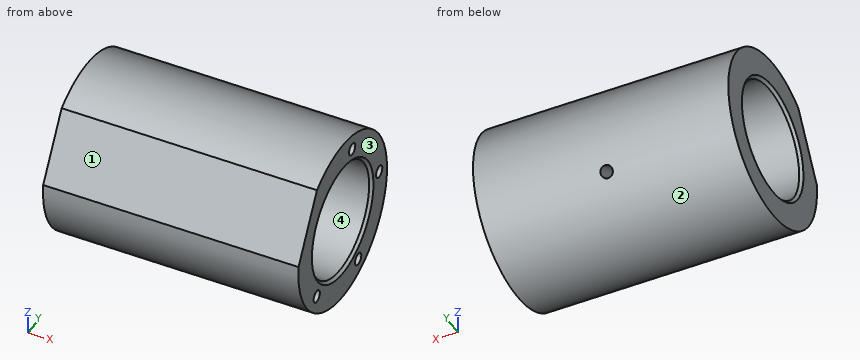
from build123d import *

# Parameters (mm, degrees)
SKETCH1_R               = 60.5
SKETCH1_R_2             = 40
BOSS_EXTRUDE1_DEPTH     = 90
CUT_EXTRUDE1_DEPTH      = 125.179305844
CUT_EXTRUDE1_DEPTH_BACK = 125.179305844
SKETCH6_W               = 4.25
SKETCH6_H               = 82.644536929
M10_TAPPED_HOLE2_D      = 8.5
M10_TAPPED_HOLE2_DEPTH  = 32
M10_TAPPED_HOLE2_TIP    = 2.553657631
CHAMFER1_SIZE           = 2


with BuildPart() as part:
    # Sketch1 → Boss-Extrude1 (new, symmetric)
    with BuildSketch(Plane(origin=(0, 0, 0), x_dir=(0, 0, -1), z_dir=(1, 0, 0))):
        with Locations(Location((0, 0, 0), (0, 0, 180))):
            Circle(SKETCH1_R)
        with Locations(Location((0, 0, 0), (0, 0, 180))):
            Circle(SKETCH1_R_2, mode=Mode.SUBTRACT)
    extrude(amount=BOSS_EXTRUDE1_DEPTH, both=True)

    # Sketch5 → Cut-Extrude1 (cut, two sides: drawn at the far end of the back side and taken through both)
    with BuildSketch(Plane(origin=(0, 0, 0), x_dir=(0, 0, -1), z_dir=(1, 0, 0)).offset(-CUT_EXTRUDE1_DEPTH_BACK)):
        with BuildLine():
            Line((-49.327448316, -35.029314047), (-5.672551684, -60.233480369))
            ThreePointArc((-5.672551684, -60.233480369), (-30.25, -52.394536929), (-49.327448316, -35.029314047))
        make_face()
    extrude(amount=CUT_EXTRUDE1_DEPTH + CUT_EXTRUDE1_DEPTH_BACK, mode=Mode.SUBTRACT)

    # Sketch6 → M10 Tapped Hole1 (revolve, cut)
    with BuildSketch(Plane(origin=(0, 0, 0), x_dir=(0, -0.500000000000001, -0.8660254037844382), z_dir=(1, 0, 0))):
        with Locations((2.125, 41.322268465)):
            Rectangle(SKETCH6_W, SKETCH6_H)
    revolve(axis=Axis((0, -5.499261314, 3.175), (0, 0.866025403784438, -0.500000000000001)), mode=Mode.SUBTRACT)

    # M10 Tapped Hole2
    with Locations(Plane(origin=(90, 0, 0), x_dir=(0, 0, -1), z_dir=(1, 0, 0))):
        with Locations((-4.357787137, 49.809734905), (45.315389352, 21.130913087), (35.355339059, -35.355339059), (-48.296291314, 12.940952255)):
            Hole(M10_TAPPED_HOLE2_D / 2, depth=M10_TAPPED_HOLE2_DEPTH)
            with Locations((0, 0, -(M10_TAPPED_HOLE2_DEPTH + M10_TAPPED_HOLE2_TIP / 2))):  # 118° drill point
                Cone(0, M10_TAPPED_HOLE2_D / 2, M10_TAPPED_HOLE2_TIP, mode=Mode.SUBTRACT)

    # Chamfer1
    chamfer1_edges = [part.edges().sort_by_distance(p)[0] for p in [
        (-90, 0, -40),
        (90, 0, -40),
    ]]
    chamfer(chamfer1_edges, length=CHAMFER1_SIZE)


solid = part.part
Can you work these out from the model? Positions are in its coordinate system, mm. Face numbers are marked on the shaded views. Give positions to 0.01 mm unless a question says otherwise; leave off trailing zeros. Loops run counter-clockwise (first coordinate to the right, second up) from the corner with the lowest first, then second, coordinate; pieces in that order, holes last. Notation, with made-up numbers: (61.5, 40) - (71.5, 40) arc R20 ccw to (71.5, 66) - close; hole circle Ø2 at (-28, 35). An arc over 180 degrees is marked (long way). Return JSON: item names as keys, results as strings.
1. I'm going to push flat-ended pins straight in: pin 1 Ø12 at (x, z) = (-30.5, 23) entering from +Y; pin 2 Ø4 at (x, z) = (-46, 37) entering from +Y; pin 3 Ø12 at (x, z) = (19, -40) entering from +Y. Where does each tip first touch, or does it pass through?
Output values:
{"pin 1": "stops at y = 58.06", "pin 2": "stops at y = 49.35", "pin 3": "stops at y = 50.04"}
2. I want a section at C-C on x = 79. Please give me the cut outline in (y, z).
Output values:
{"outline": "(-60.23, 5.67) arc R60.5 ccw (long way) to (-35.03, 49.33) - close; hole circle Ø80 at (0, 0); hole circle Ø8.5 at (-35.36, -35.36); hole circle Ø8.5 at (12.94, 48.3); hole circle Ø8.5 at (21.13, -45.32); hole circle Ø8.5 at (49.81, 4.36)"}
3. We'd pull the mould along Z, two halves only. Please class the marked faces 1, 2, 3 and 4: +Z half, -Z half, draft (parallel to the pull), parting line (faces both ways), or undercut.
Output values:
{"face 1": "+Z half", "face 2": "parting line", "face 3": "draft", "face 4": "undercut"}
4. I want a section at B-B on x = -11. Please give me the cut outline in (y, z).
Output values:
{"outline": "(-60.23, 5.67) arc R60.5 ccw (long way) to (-35.03, 49.33) - close; hole circle Ø80 at (0, 0)"}
5. I want a section at A-A on y = 0. Please give me the cut outline in (x, z).
Output values:
{"outline": "(-90, -60.5) - (90, -60.5) - (90, -42) - (88, -40) - (-88, -40) - (-90, -42) - close; (-90, 42) - (-88, 40) - (88, 40) - (90, 42) - (90, 60.5) - (-90, 60.5) - close"}
6. If I drill on line 1 (Z direction, x = 61, y = -35); line 2 (Y direction, x = 54, z = -5.5); line 3 (Z direction, x = 1.5, y = 1.5), over which ranges is the centre line in solid material (lowest first)?
Output values:
{"line 1": "z = -49.35 to -39.59, -31.12 to -19.36, 19.36 to 49.35", "line 2": "y = -60.25 to -39.62, 39.62 to 60.25", "line 3": "z = -60.48 to -39.97, 39.97 to 60.48"}
